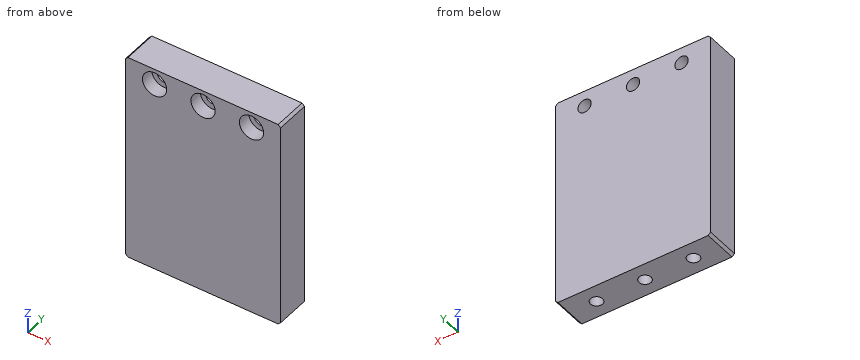
from build123d import *

# Parameters (mm, degrees)
SKETCH_1_W                  = 64
SKETCH_1_H                  = 14
EXTRUDE_1_DEPTH             = 87
HOLE_WIZARD_C_0_D           = 5.5
HOLE_WIZARD_C_0_CBORE_D     = 10
HOLE_WIZARD_C_0_CBORE_DEPTH = 5.5
HOLE_WIZARD_M6_1_D          = 5
HOLE_WIZARD_M6_1_DEPTH      = 13.5
HOLE_WIZARD_M6_1_TIP        = 1.502151548
CHAMFER_1_SIZE              = 1


with BuildPart() as part:
    # 草图1 → 凸台-拉伸1 (new body)
    with BuildSketch(Plane.XY):
        with Locations((10, -67.679969714)):
            Rectangle(SKETCH_1_W, SKETCH_1_H)
    extrude(amount=EXTRUDE_1_DEPTH)

    # 打孔尺寸根据六角头螺栓 C 级的类型0 (through all)
    with Locations(Plane(origin=(0, -74.679969714, 0), x_dir=(-1, 0, 0), z_dir=(0, -1, 0))):
        with Locations((10, -80.5), (-10, -80.5), (-30, -80.5)):
            CounterBoreHole(HOLE_WIZARD_C_0_D / 2, HOLE_WIZARD_C_0_CBORE_D / 2, HOLE_WIZARD_C_0_CBORE_DEPTH)

    # M6 螺纹孔1
    with Locations(Plane(origin=(0, 0, 0), x_dir=(-1, 0, 0), z_dir=(0, 0, -1))):
        with Locations((-30, -67.679969714), (-10, -67.679969714), (10, -67.679969714)):
            Hole(HOLE_WIZARD_M6_1_D / 2, depth=HOLE_WIZARD_M6_1_DEPTH)
            with Locations((0, 0, -(HOLE_WIZARD_M6_1_DEPTH + HOLE_WIZARD_M6_1_TIP / 2))):  # 118° drill point
                Cone(0, HOLE_WIZARD_M6_1_D / 2, HOLE_WIZARD_M6_1_TIP, mode=Mode.SUBTRACT)

    # 倒角1
    chamfer_1_edges = [part.edges().sort_by_distance(p)[0] for p in [
        (42, -67.679969714, 87),
        (-22, -67.679969714, 87),
        (42, -67.679969714, 0),
        (-22, -67.679969714, 0),
    ]]
    chamfer(chamfer_1_edges, length=CHAMFER_1_SIZE)


solid = part.part
Here's how the part is built. I have some questions about the finished solid (model axes, mm). Round coordinates to 2 decimals unless told otherwise and drop trailing zeros. Write each loop counter-clockwise with the first axis right and the second up, starting at its lowest first coordinate (ties: lowest second). Pieces come first, ordered by that corner, then holes.
1. Suppose I cut it at B-B (z = 7). List the corners of the cut face in (x, y) for me, and give its area (3 significant figures).
2. Will these pins go through, and if not, where does the flat tip stop? pin 1 Ø4.5 at (x, y) = (10, -67.68) entering from -Z; pin 2 Ø9 at (x, z) = (-10, 80.5) entering from +Y; pin 3 Ø4 at (x, y) = (30, -67.68) entering from -Z; pin 4 Ø8 at (x, z) = (10.5, 80) entering from -Y.
3. I need wall thicknesses on L1, parallel to X at y = -66.5, z = 80.5; L2, parallel to X at y = -71.2, z = 80.5; L3, parallel to Y at x = 30, z = 5.75. Which ranges of each line are inside material? Lowest first, please.
4. Suppose I cut it at A-A (z = 80.5). List the corners of the cut face in (x, y) for me.
Answer sheet:
1. outline: (-22, -74.68) - (42, -74.68) - (42, -60.68) - (-22, -60.68) - close; hole circle Ø5 at (-10, -67.68); hole circle Ø5 at (10, -67.68); hole circle Ø5 at (30, -67.68)
1. area: 837 mm2
2. pin 1: stops at z = 13.65
2. pin 2: stops at y = -60.68
2. pin 3: stops at z = 13.8
2. pin 4: stops at y = -69.18
3. L1: x = -22 to -12.75, -7.25 to 7.25, 12.75 to 27.25, 32.75 to 42
3. L2: x = -22 to -15, -5 to 5, 15 to 25, 35 to 42
3. L3: y = -74.68 to -70.18, -65.18 to -60.68
4. outline: (-22, -74.68) - (-15, -74.68) - (-15, -69.18) - (-12.75, -69.18) - (-12.75, -60.68) - (-22, -60.68) - close; (-7.25, -69.18) - (-5, -69.18) - (-5, -74.68) - (5, -74.68) - (5, -69.18) - (7.25, -69.18) - (7.25, -60.68) - (-7.25, -60.68) - close; (12.75, -69.18) - (15, -69.18) - (15, -74.68) - (25, -74.68) - (25, -69.18) - (27.25, -69.18) - (27.25, -60.68) - (12.75, -60.68) - close; (32.75, -69.18) - (35, -69.18) - (35, -74.68) - (42, -74.68) - (42, -60.68) - (32.75, -60.68) - close
